```python
from build123d import *

# Parameters (mm, degrees)
BOSS_EXTRUDE1_DEPTH = 10
SKETCH2_R           = 13
CUT_EXTRUDE1_DEPTH  = 140.620915339


with BuildPart() as part:
    # Sketch1 → Boss-Extrude1 (new body)
    with BuildSketch(Plane.XY):
        with BuildLine():
            Line((-25, 0), (-25, 137))
            Line((-25, 137), (25, 137))
            Line((25, 137), (25, 0))
            ThreePointArc((25, 0), (0, -25), (-25, 0))
        make_face()
    extrude(amount=BOSS_EXTRUDE1_DEPTH)

    # Sketch2 → Cut-Extrude1 (cut, through all)
    with BuildSketch(Plane.XY.offset(10)):
        with Locations((0, -8)):
            Circle(SKETCH2_R)
    extrude(amount=-CUT_EXTRUDE1_DEPTH, mode=Mode.SUBTRACT)


solid = part.part
```
Work out the finished part from the listing and answer in its coordinate system (mm). Coordinates: 2 decimals unless noted, no trailing zeros. Write each loop counter-clockwise with the first axis right and the second up, starting at its lowest first coordinate (ties: lowest second). Pieces come first, ordered by that corner, then holes.
Q1. A cutting plane is placed at D-D, the plane x = -19.5. Give the vertices of the cut face in (y, z), then the cut area to 3 significant figures.
Q2. Each of these flat-tipped pins is pushed along its axis until it touches: pin 1 Ø1.5 at (x, y) = (-15.5, 77.5) entering from -Z; pin 2 Ø1.5 at (x, z) = (-1, 6) entering from -Y; pin 3 Ø1.5 at (x, z) = (-10, 7.5) entering from -Y; pin 4 Ø15.5 at (x, y) = (0, -8) entering from +Z. Where does it stop, or does it pass through?
Q3. A cutting plane is placed at A-A, the plane x = 0. Give the vertices of the cut face in (y, z), then the cut area to 3 significant figures.
Q4. A cutting plane is placed at B-B, the plane z = 5. Give the vertices of the cut face in (x, y), then the cut area to 3 significant figures.
Q5. A cutting plane is placed at C-C, the plane y = -8. Give the vertices of the cut face in (x, z), then the cut area to 3 significant figures.
Q6. Determine the mould class of faces 1 (the face through (0, 57, 10)), 2 (the face through (-10.316, -15.91, 5.07)), 3 (the face through (0, 137, 5)) for opening direction Y: released by +Y, released by -Y, zero draft, split by the parting line, or undercut.
Q7. Find the intervals of material crossed by line 1 (Y direction, x = 0, z = 3.25); line 2 (Y direction, x = -10.5, z = 1.5); line 3 (Y direction, x = -14, z = 7.25), in increasing order.
Findings below:
1. outline: (-15.64, 0) - (137, 0) - (137, 10) - (-15.64, 10) - close
1. area: 1,530 mm2
2. pin 1: stops at z = 0
2. pin 2: stops at y = -25
2. pin 3: stops at y = -23.23
2. pin 4: passes through
3. outline: (-25, 0) - (-21, 0) - (-21, 10) - (-25, 10) - close; (5, 0) - (137, 0) - (137, 10) - (5, 10) - close
3. area: 1,360 mm2
4. outline: (-25, 0) arc R25 ccw to (25, 0) - (25, 137) - (-25, 137) - close; hole circle Ø26 at (0, -8)
4. area: 7,300 mm2
5. outline: (-23.69, 0) - (-13, 0) - (-13, 10) - (-23.69, 10) - close; (13, 0) - (23.69, 0) - (23.69, 10) - (13, 10) - close
5. area: 214 mm2
6. face 1: zero draft
6. face 2: undercut
6. face 3: released by +Y
7. line 1: y = -25 to -21, 5 to 137
7. line 2: y = -22.69 to -15.66, -0.34 to 137
7. line 3: y = -20.71 to 137
